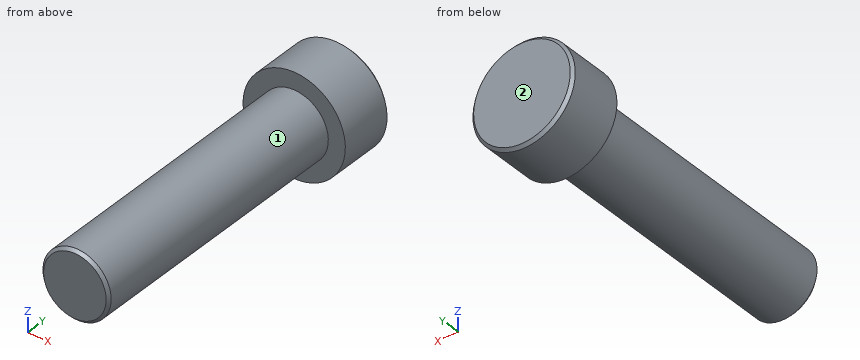
from build123d import *

# Parameters (mm, degrees)
SKETCH_1_R      = 6
EXTRUDE_1_DEPTH = 25
SKETCH_2_R      = 9
EXTRUDE_2_DEPTH = 10
CHAMFER_1_SIZE  = 0.5


with BuildPart() as part:
    # 草图1 → 凸台-拉伸1 (new, symmetric)
    with BuildSketch(Plane(origin=(0, 0, 0), x_dir=(1, 0, 0), z_dir=(0, 1, 0))):
        with Locations(Location((0, 0, 0), (0, 0, 270))):
            Circle(SKETCH_1_R)
    extrude(amount=EXTRUDE_1_DEPTH, both=True)

    # 草图2 → 凸台-拉伸2 (add)
    with BuildSketch(Plane(origin=(0, 25, 0), x_dir=(1, 0, 0), z_dir=(0, 1, 0))):
        with Locations(Location((0, 0, 0), (0, 0, 270))):
            Circle(SKETCH_2_R)
    extrude(amount=EXTRUDE_2_DEPTH)

    # 倒角1
    chamfer_1_edges = [part.edges().sort_by_distance(p)[0] for p in [
        (0, -25, -6),
        (0, 35, -9),
    ]]
    chamfer(chamfer_1_edges, length=CHAMFER_1_SIZE)


solid = part.part
Geometry: final body of the model. Coordinates: model frame, mm. Face numbers are marked on the shaded views. A direction names the side the tool comes from. Give positions to 0.01 mm unless a question says otherwise; leave off trailing zeros. Write each loop counter-clockwise with the first axis right and the second up, starting at its lowest first coordinate (ties: lowest second). Pieces come first, ordered by that corner, then holes.
(1) Cut plane A-A, the plane x = 0. Return loops of the section in (y, z).
(2) Access query for the marked faces 1 and 2. Directions: +Z, -Z, +X, -X, +Y, -Y. A direction counts if a zero-diameter tool reaches every point of the face in a straight line with its end or side. Return the directions, or none.
(3) Cut plane D-D, the plane y = 19. Return loops of the section in (x, z).
(4) Ray query, line 1 (Y direction, x = -6.5, z = -0.5); line 2 (Z direction, x = 0.75, y = 9); line 3 (X direction, y = 3, z = -0.5). Return the intervals inside material, ascending.
(5) Cut plane B-B, the plane z = 0. Return loops of the section in (x, y).
(6) First-contact query: P1, Ø1.5, axis at x = -3, y = 25.5, coming from the +Z side; P2, Ø8, axis at y = 15, z = -5.5, coming from the -X side; P3, Ø4, axis at y = 16, z = 5.5, coming from the +X side. Flat tips, straight axial feed; report the tip coordinate or a pass-through.
(7) Cut plane C-C, the plane y = 31.5. Return loops of the section in (x, z).
Values follow:
1. outline: (-25, -5.5) - (-24.5, -6) - (25, -6) - (25, -9) - (34.5, -9) - (35, -8.5) - (35, 8.5) - (34.5, 9) - (25, 9) - (25, 6) - (-24.5, 6) - (-25, 5.5) - close
2. face 1: -Y
2. face 2: +Z, -Z, +X, -X, +Y
3. outline: circle Ø12 at (0, 0)
4. line 1: y = 25 to 35
4. line 2: z = -5.95 to 5.95
4. line 3: x = -5.98 to 5.98
5. outline: (-9, 25) - (-6, 25) - (-6, -24.5) - (-5.5, -25) - (5.5, -25) - (6, -24.5) - (6, 25) - (9, 25) - (9, 34.5) - (8.5, 35) - (-8.5, 35) - (-9, 34.5) - close
6. P1: stops at z = 8.71
6. P2: stops at x = -5.81
6. P3: stops at x = 4.87
7. outline: circle Ø18 at (0, 0)
